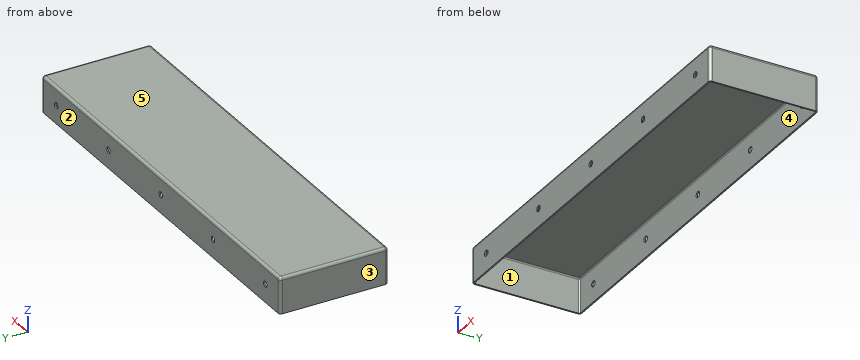
```python
from build123d import *

# Parameters (mm, degrees)
SKETCH_1_W         = 455
SKETCH_1_H         = 120
EXTRUDE_1_DEPTH    = 40
FILLET_1_R         = 3
SHELL_1_T          = -1.5
HOLE_WIZARD_M6_1_D = 6.6


with BuildPart() as part:
    # 草图1 → 凸台-拉伸1 (new body)
    with BuildSketch(Plane.XY):
        Rectangle(SKETCH_1_W, SKETCH_1_H)
    extrude(amount=EXTRUDE_1_DEPTH)

    # 圆角1
    fillet_1_edges = [part.edges().sort_by_distance(p)[0] for p in [
        (-227.5, 0, 40),
        (0, -60, 40),
        (227.5, 0, 40),
        (0, 60, 40),
        (227.5, -60, 20),
        (-227.5, -60, 20),
        (-227.5, 60, 20),
        (227.5, 60, 20),
    ]]
    fillet(fillet_1_edges, radius=FILLET_1_R)

    # 抽壳1
    shell_1_openings = [part.faces().sort_by_distance(p)[0] for p in [
        (0, 0, 0),
    ]]
    offset(amount=SHELL_1_T, openings=shell_1_openings, kind=Kind.INTERSECTION)

    # M6 间隙孔1 (through all)
    with Locations(Plane(origin=(0, -60, 0), x_dir=(-1, 0, 0), z_dir=(0, -1, 0))):
        with Locations((200, -20), (100, -20), (-100, -20), (-200, -20), (0, -20)):
            Hole(HOLE_WIZARD_M6_1_D / 2)


solid = part.part
```
Geometry check sheet. Reference: the model listing, model coordinates, mm. Face numbers are marked on the shaded views. A direction names the side the tool comes from. Give positions to 0.01 mm unless a question says otherwise; leave off trailing zeros. Order: outer loops, then holes, each group sorted by start corner. A loop starts at its lowest first (then second) coordinate and runs counter-clockwise, first axis right, second up.
1. Section check C-C, the plane x = 163. Enter the section's corners in (y, z), and give its area (3 significant figures).
2. Section check B-B, the plane z = 33. Enter the section's corners in (x, y), and give its area (3 significant figures).
3. Section check A-A, the plane y = -26. Enter the section's corners in (x, z).
4. Gauge pin test, flat ends, axial feed: pin 1 Ø4 at (x, y) = (5, -47) entering from -Z; pin 2 Ø7.5 at (x, z) = (200, 20) entering from +Y. Record the tip position at first contact, or that the pin passes through.
5. Access from +Z, -Z, +X, -X, +Y, -Y to the whole of each face (thin tool, end or side, straight path). Record for the marked faces 4 and 5.
6. Release check for a two-part mould opening along Y. For the marked faces 1, 2 and 3 record: pulls with the +Y half, pulls with the -Y half, needs draft (parallel to the pull), parting line crosses it, or undercut.
7. Thickness scan on L1, parallel to Y at x = -205, z = 32; L2, parallel to X at y = 26, z = 32; L3, parallel to Z at x = -160.5, y = 22. Record the ranges inside material, lowest first.
Values follow:
1. outline: (-60, 0) - (-58.5, 0) - (-58.5, 37) arc R1.5 cw to (-57, 38.5) - (57, 38.5) arc R1.5 cw to (58.5, 37) - (58.5, 0) - (60, 0) - (60, 37) arc R3 ccw to (57, 40) - (-57, 40) arc R3 ccw to (-60, 37) - close
1. area: 293 mm2
2. outline: (-227.5, -57) arc R3 ccw to (-224.5, -60) - (224.5, -60) arc R3 ccw to (227.5, -57) - (227.5, 57) arc R3 ccw to (224.5, 60) - (-224.5, 60) arc R3 ccw to (-227.5, 57) - close; hole (-226, -57) arc R1.5 ccw to (-224.5, -58.5) - (224.5, -58.5) arc R1.5 ccw to (226, -57) - (226, 57) arc R1.5 ccw to (224.5, 58.5) - (-224.5, 58.5) arc R1.5 ccw to (-226, 57) - close
2. area: 1,710 mm2
3. outline: (-227.5, 0) - (-226, 0) - (-226, 37) arc R1.5 cw to (-224.5, 38.5) - (224.5, 38.5) arc R1.5 cw to (226, 37) - (226, 0) - (227.5, 0) - (227.5, 37) arc R3 ccw to (224.5, 40) - (-224.5, 40) arc R3 ccw to (-227.5, 37) - close
4. pin 1: stops at z = 38.5
4. pin 2: stops at y = 60
5. face 4: -Z
5. face 5: +Z, +X, -X, +Y, -Y
6. face 1: undercut
6. face 2: pulls with the +Y half
6. face 3: needs draft
7. L1: y = -60 to -58.5, 58.5 to 60
7. L2: x = -227.5 to -226, 226 to 227.5
7. L3: z = 38.5 to 40
